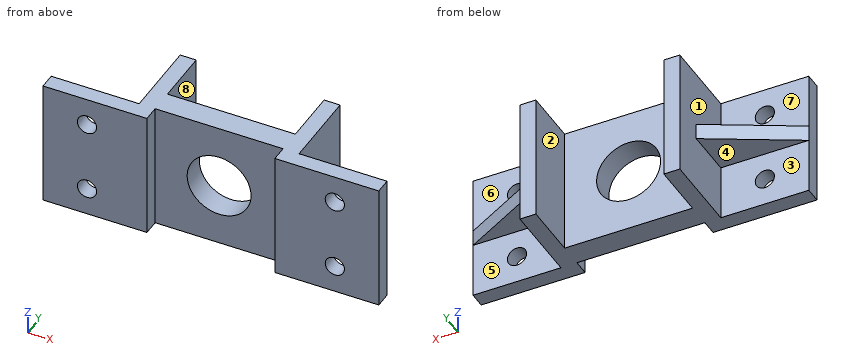
from build123d import *

# Parameters (mm, degrees)
BASE_BODY_DEPTH          = 60
CENTER_BORE_SKETCH_R     = 20
CENTER_BORE_DEPTH        = 15
GUSSET_1_BLANK_DEPTH     = 40
GUSSET_1_TRIM_A_DEPTH    = 25
GUSSET_1_TRIM_B_DEPTH    = 5
GUSSET_2_BLANK_DEPTH     = 35
GUSSET_2_TRIM_DEPTH      = 25
FLANGE_EXTENSION_1_DEPTH = 10
FLANGE_EXTENSION_2_DEPTH = 10
MOUNTING_HOLES_SKETCH_R  = 6
MOUNTING_HOLES_4X_DEPTH  = 10


with BuildPart() as part:
    # Base Profile Sketch → Base Body (new body)
    with BuildSketch(Plane.XY):
        Polygon((0, 0), (55, 0), (65, 0), (65, 10), (145, 10), (145, 0), (210, 0), (210, 10), (155, 10), (155, 60), (145, 60), (145, 25), (65, 25), (65, 60), (55, 60), (55, 10), (0, 10), align=None)
    extrude(amount=BASE_BODY_DEPTH)

    # Center Bore Sketch → Center Bore (cut)
    with BuildSketch(Plane(origin=(0, 25, 0), x_dir=(1, 0, 0), z_dir=(0, 1, 0))):
        with Locations(Location((105, -30, 0), (0, 0, 270))):
            Circle(CENTER_BORE_SKETCH_R)
    extrude(amount=-CENTER_BORE_DEPTH, mode=Mode.SUBTRACT)

    # Gusset 1 Sketch → Gusset 1 Blank (add)
    with BuildSketch(Plane.XY.offset(60)):
        Polygon((155, 10), (155, 40), (210, 10), align=None)
    extrude(amount=-GUSSET_1_BLANK_DEPTH)

    # Gusset 1 Trim A Sketch → Gusset 1 Trim A (cut)
    with BuildSketch(Plane.XY.offset(60)):
        Polygon((155, 40), (155, 10), (210, 10), align=None)
    extrude(amount=-GUSSET_1_TRIM_A_DEPTH, mode=Mode.SUBTRACT)

    # Gusset 1 Trim B Sketch → Gusset 1 Trim B (cut)
    with BuildSketch(Plane(origin=(0, 0, 20), x_dir=(-1, 0, 0), z_dir=(0, 0, -1))):
        Polygon((-210, 10), (-155, 10), (-155, 40), align=None)
    extrude(amount=-GUSSET_1_TRIM_B_DEPTH, mode=Mode.SUBTRACT)

    # Gusset 2 Sketch → Gusset 2 Blank (add)
    with BuildSketch(Plane(origin=(0, 0, 0), x_dir=(-1, 0, 0), z_dir=(0, 0, -1))):
        Polygon((-55, 10), (-55, 40), (0, 10), align=None)
    extrude(amount=-GUSSET_2_BLANK_DEPTH)

    # Gusset 2 Trim Sketch → Gusset 2 Trim (cut)
    with BuildSketch(Plane(origin=(0, 0, 0), x_dir=(-1, 0, 0), z_dir=(0, 0, -1))):
        Polygon((-55, 40), (-55, 10), (0, 10), align=None)
    extrude(amount=-GUSSET_2_TRIM_DEPTH, mode=Mode.SUBTRACT)

    # Flange Extension 1 Sketch → Flange Extension 1 (add)
    with BuildSketch(Plane.XY.offset(60)):
        Polygon((0, 0), (0, 10), (55, 10), (55, 60), (65, 60), (65, 25), (145, 25), (145, 60), (155, 60), (155, 10), (210, 10), (210, 0), (145, 0), (145, 10), (65, 10), (65, 0), align=None)
    extrude(amount=FLANGE_EXTENSION_1_DEPTH)

    # Flange Extension 2 Sketch → Flange Extension 2 (add)
    with BuildSketch(Plane(origin=(0, 0, 0), x_dir=(-1, 0, 0), z_dir=(0, 0, -1))):
        Polygon((-210, 0), (-210, 10), (-155, 10), (-155, 60), (-145, 60), (-145, 25), (-65, 25), (-65, 60), (-55, 60), (-55, 10), (0, 10), (0, 0), (-65, 0), (-65, 10), (-145, 10), (-145, 0), align=None)
    extrude(amount=FLANGE_EXTENSION_2_DEPTH)

    # Mounting Holes Sketch → Mounting Holes 4x (cut)
    with BuildSketch(Plane(origin=(0, 10, 0), x_dir=(1, 0, 0), z_dir=(0, 1, 0))):
        with Locations(Location((27.5, -52.5, 0), (0, 0, 270))):
            Circle(MOUNTING_HOLES_SKETCH_R)
        with Locations(Location((27.5, -7.5, 0), (0, 0, 270))):
            Circle(MOUNTING_HOLES_SKETCH_R)
        with Locations(Location((182.5, -7.5, 0), (0, 0, 270))):
            Circle(MOUNTING_HOLES_SKETCH_R)
        with Locations(Location((182.5, -52.5, 0), (0, 0, 270))):
            Circle(MOUNTING_HOLES_SKETCH_R)
    extrude(amount=-MOUNTING_HOLES_4X_DEPTH, mode=Mode.SUBTRACT)


solid = part.part
Source: CAD feature listing. Evaluate the final solid. Frame: model axes, mm. Face numbers are marked on the shaded views. A direction names the side the tool comes from. Coordinates: 2 decimals unless noted, no trailing zeros. Loops run counter-clockwise (first coordinate to the right, second up) from the corner with the lowest first, then second, coordinate; pieces in that order, holes last. Notation, with made-up numbers: (58, -19) -> (102, -19) arc R26 cw to (102, 1) -> close; hole circle Ø5 at (-25, 21). An arc over 180 degrees is marked (long way). Answer in a Markdown table with one row per item. Add a question column.
Q1. Section C-C on z = 30. Return the cut outline in (x, y), and give its area (3 significant figures).
Q2. Section A-A on y = 8. Return the cut outline in (x, z), and give its area (3 significant figures).
Q3. Section D-D on y = 42.5. Return the cut outline in (x, z), and give its area (3 significant figures).
Q4. Reachability of the marked faces 4, 5, 6, 7 and 8 from +Z, -Z, +X, -X, +Y, -Y: full face, straight path, thin tool, end or side. Return the list, or none.
Q5. Ray query, line 1 along X through (y, z) = (3.5, 52.5); line 2 along X through (y, z) = (41.5, 25.5); line 3 along Y through (x, z) = (67, 3). Return the intervals inside material, ascending.
Q6. Pull-direction query (X, two-part tool) for the marked faces 1, 2 and 3; classes: pulls with the +X half, pulls with the -X half, needs draft (parallel to the pull), parting line crosses it, or undercut.
Q7. Contact query for flat-ended pins moving along their axis: pin 1 Ø9.5 at (x, z) = (27.5, 52.5) entering from -Y; pin 2 Ø11 at (y, z) = (5, 30) entering from -X; pin 3 Ø17.5 at (x, z) = (193, 50) entering from +Y; pin 4 Ø1 at (x, z) = (86, 56) entering from +Y. Output: stop coordinate, or through.
Q8. Section B-B on x = 105. Return the cut outline in (y, z).
Computed values:
| question | item | result |
|---|---|---|
| 1 | outline | (0, 0) -> (65, 0) -> (65, 10) -> (85, 10) -> (85, 25) -> (65, 25) -> (65, 60) -> (55, 60) -> (55, 40) -> (0, 10) -> close; (125, 10) -> (145, 10) -> (145, 0) -> (210, 0) -> (210, 10) -> (155, 40) -> (155, 60) -> (145, 60) -> (145, 25) -> (125, 25) -> close |
| 1 | area | 4,550 mm^2 |
| 2 | outline | (0, -10) -> (65, -10) -> (65, 70) -> (0, 70) -> close; (145, -10) -> (210, -10) -> (210, 70) -> (145, 70) -> close; hole circle Ø12 at (27.5, 7.5); hole circle Ø12 at (27.5, 52.5); hole circle Ø12 at (182.5, 7.5); hole circle Ø12 at (182.5, 52.5) |
| 2 | area | 9,950 mm^2 |
| 3 | outline | (55, -10) -> (65, -10) -> (65, 70) -> (55, 70) -> close; (145, -10) -> (155, -10) -> (155, 70) -> (145, 70) -> close |
| 3 | area | 1,600 mm^2 |
| 4 | face 4 | -Z, -X, +Y |
| 4 | face 5 | -Z, +X, +Y |
| 4 | face 6 | +Z, +X, +Y |
| 4 | face 7 | +Z, -X, +Y |
| 4 | face 8 | +Z, -Z, +Y |
| 5 | line 1 | x = 0 to 21.5, 33.5 to 65, 145 to 176.5, 188.5 to 210 |
| 5 | line 2 | x = 55 to 65, 145 to 155 |
| 5 | line 3 | y = 10 to 25 |
| 6 | face 1 | pulls with the -X half |
| 6 | face 2 | undercut |
| 6 | face 3 | needs draft |
| 7 | pin 1 | passes through |
| 7 | pin 2 | stops at x = 0 |
| 7 | pin 3 | stops at y = 10 |
| 7 | pin 4 | stops at y = 25 |
| 8 | outline | (10, -10) -> (25, -10) -> (25, 10) -> (10, 10) -> close; (10, 50) -> (25, 50) -> (25, 70) -> (10, 70) -> close |
